```python
from build123d import *

# Parameters (mm, degrees)
SKETCH1_R           = 175
SKETCH1_R_2         = 30
BOSS_EXTRUDE1_DEPTH = 220
BOSS_EXTRUDE2_START = -15
SKETCH2_R           = 200
SKETCH2_R_2         = 4.5
SKETCH2_R_3         = 30
BOSS_EXTRUDE2_DEPTH = 15
SKETCH3_R           = 160
SKETCH3_R_2         = 45
CUT_EXTRUDE1_DEPTH  = 200
SKETCH4_R           = 30
BOSS_EXTRUDE3_DEPTH = 20
SKETCH7_W           = 18
SKETCH7_H           = 20.211896708
CUT_EXTRUDE2_DEPTH  = 200


with BuildPart() as part:
    # Sketch1 → Boss-Extrude1 (new body)
    with BuildSketch(Plane.XY):
        Circle(SKETCH1_R)
        Circle(SKETCH1_R_2, mode=Mode.SUBTRACT)
    extrude(amount=BOSS_EXTRUDE1_DEPTH)

    # Sketch2 → Boss-Extrude2 (add)
    with BuildSketch(Plane.XY.offset(220).offset(BOSS_EXTRUDE2_START)):
        Circle(SKETCH2_R)
        with Locations((0, 190)):
            Circle(SKETCH2_R_2, mode=Mode.SUBTRACT)
        with Locations((111.679197936, 153.713228931)):
            Circle(SKETCH2_R_2, mode=Mode.SUBTRACT)
        with Locations((180.700738096, 58.713228931)):
            Circle(SKETCH2_R_2, mode=Mode.SUBTRACT)
        with Locations((180.700738096, -58.713228931)):
            Circle(SKETCH2_R_2, mode=Mode.SUBTRACT)
        with Locations((111.679197936, -153.713228931)):
            Circle(SKETCH2_R_2, mode=Mode.SUBTRACT)
        with Locations((0, -190)):
            Circle(SKETCH2_R_2, mode=Mode.SUBTRACT)
        with Locations((-111.679197936, -153.713228931)):
            Circle(SKETCH2_R_2, mode=Mode.SUBTRACT)
        with Locations((-180.700738096, -58.713228931)):
            Circle(SKETCH2_R_2, mode=Mode.SUBTRACT)
        with Locations((-180.700738096, 58.713228931)):
            Circle(SKETCH2_R_2, mode=Mode.SUBTRACT)
        with Locations((-111.679197936, 153.713228931)):
            Circle(SKETCH2_R_2, mode=Mode.SUBTRACT)
        Circle(SKETCH2_R_3, mode=Mode.SUBTRACT)
    extrude(amount=BOSS_EXTRUDE2_DEPTH)

    # Sketch3 → Cut-Extrude1 (cut)
    with BuildSketch(Plane.XY.offset(220)):
        Circle(SKETCH3_R)
        Circle(SKETCH3_R_2, mode=Mode.SUBTRACT)
    extrude(amount=-CUT_EXTRUDE1_DEPTH, mode=Mode.SUBTRACT)

    # Sketch4 → Boss-Extrude3 (add)
    with BuildSketch(Plane(origin=(0, 0, 0), x_dir=(-1, 0, 0), z_dir=(0, 0, -1))):
        Circle(SKETCH4_R)
    extrude(amount=-BOSS_EXTRUDE3_DEPTH)

    # Sketch7 → Cut-Extrude2 (cut)
    with BuildSketch(Plane.XY.offset(220)):
        with Locations((0, 24.894051646)):
            Rectangle(SKETCH7_W, SKETCH7_H)
    extrude(amount=-CUT_EXTRUDE2_DEPTH, mode=Mode.SUBTRACT)


solid = part.part
```
Geometry check sheet. Reference: the model listing, model coordinates, mm. A direction names the side the tool comes from. Give positions to 0.01 mm unless a question says otherwise; leave off trailing zeros. Order: outer loops, then holes, each group sorted by start corner. A loop starts at its lowest first (then second) coordinate and runs counter-clockwise, first axis right, second up. Notation, with made-up numbers: (-6.5, 45.25) - (35.5, 45.25) arc R23 ccw to (35.5, 77.25) - close; hole circle Ø4 at (20, -6.5). An arc over 180 degrees is marked (long way). Write item = value, one per line. Start each with the question number.
1) Section check C-C (y = 0). Enter the section's corners in (x, z), then the cut area to 4 significant figures.
2) Scan lines: L1, parallel to Y at x = -0.5, z = 204.5; L2, parallel to Y at x = 36, z = 130.5; L3, parallel to X at y = -25.5, z = 55. Record each from-to range of solid material in increasing order.
3) Section check B-B (x = 93). Enter the section's corners in (y, z).
4) Section check A-A (z = 160.5). Enter the section's corners in (x, y), then the cut area to 3 significant figures.
5) Section check D-D (y = -166). Enter the section's corners in (x, z), then the cut area to 3 significant figures.
6) Draft check along Y on faces 1 (the cylindrical face through (-34.685, -156.195, 121.4)), 2 (the cylindrical face through (-128.982, 118.273, 101.065)), 3 (the flat face through (2, 2, 0)). Enter one of: released by +Y, released by -Y, zero draft, split by the parting line, or undercut.
7) Access from +Z, -Z, +X, -X, +Y, -Y to the whole of each face (thin tool, end or side, straight path). Record for faces 4 (the flat face through (-134, -88, 220)), 5 (the flat face through (33, -33, 20)), 6 (the flat face through (177, 1, 205)).
8) Gauge pin test, flat ends, axial feed: pin 1 Ø14.5 at (x, y) = (111.68, -153.71) entering from -Z; pin 2 Ø11.5 at (x, y) = (-111.68, 153.71) entering from +Z; pin 3 Ø7 at (y, z) = (33, 138.5) entering from +X; pin 4 Ø1 at (y, z) = (-59.5, 128) entering from -X. Record the tip position at first contact, or that the pin passes through.
Geometry check:
q1.outline = (-200, 205) - (-175, 205) - (-175, 0) - (175, 0) - (175, 205) - (200, 205) - (200, 220) - (160, 220) - (160, 20) - (45, 20) - (45, 220) - (30, 220) - (30, 20) - (-30, 20) - (-30, 220) - (-45, 220) - (-45, 20) - (-160, 20) - (-160, 220) - (-200, 220) - close
q1.area = 19,750 mm2
q2.L1 = -175 to -160, -45 to -30, 35 to 45, 160 to 175
q2.L2 = -171.26 to -155.9, -27 to 27, 155.9 to 171.26
q2.L3 = -173.13 to -157.95, -37.08 to -15.8, 15.8 to 37.08, 157.95 to 173.13
q3.outline = (-177.06, 205) - (-148.24, 205) - (-148.24, 0) - (148.24, 0) - (148.24, 205) - (177.06, 205) - (177.06, 220) - (130.2, 220) - (130.2, 20) - (-130.2, 20) - (-130.2, 220) - (-177.06, 220) - close
q4.outline = circle Ø350 at (0, 0); circle Ø90 at (0, 0); hole circle Ø320 at (0, 0); hole (-9, 28.62) arc R30 ccw (long way) to (9, 28.62) - (9, 35) - (-9, 35) - close
q4.area = 19,200 mm2
q5.outline = (-111.55, 205) - (-55.4, 205) - (-55.4, 0) - (55.4, 0) - (55.4, 205) - (111.55, 205) - (111.55, 220) - (-111.55, 220) - close
q5.area = 26,100 mm2
q6.face_1 = undercut
q6.face_2 = split by the parting line
q6.face_3 = zero draft
q7.face_4 = +Z, +X, -X, +Y, -Y
q7.face_5 = +Z
q7.face_6 = -Z
q8.pin_1 = 205
q8.pin_2 = 220
q8.pin_3 = 172.5
q8.pin_4 = -164.75
